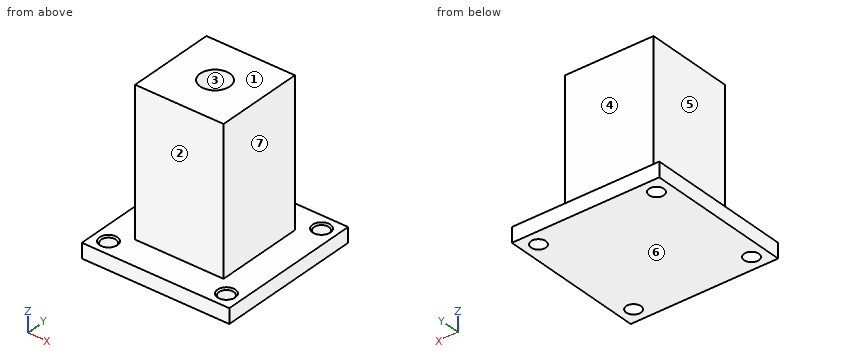
```python
from build123d import *

# Parameters (mm, degrees)
SKETCH_1_W                   = 30
SKETCH_1_H                   = 30
EXTRUDE_1_DEPTH              = 54
SKETCH_2_W                   = 50
SKETCH_2_H                   = 50
EXTRUDE_2_DEPTH              = 5
HOLE_WIZARD_M6_1_D           = 5
HOLE_WIZARD_M6_1_DEPTH       = 13.497848452
HOLE_WIZARD_M6_1_CSINK_D     = 6.05
HOLE_WIZARD_M6_1_CSINK_ANGLE = 90
HOLE_WIZARD_M6_1_TIP         = 1.502151548
SKETCH_6_R                   = 5
CUT_EXTRUDE_1_DEPTH          = 39


with BuildPart() as part:
    # 草图1 → 凸台-拉伸1 (new body)
    with BuildSketch(Plane.XY):
        with Locations((-50, 0)):
            Rectangle(SKETCH_1_W, SKETCH_1_H)
    extrude(amount=EXTRUDE_1_DEPTH)

    # 草图2 → 凸台-拉伸2 (add)
    with BuildSketch(Plane.XY):
        with Locations((-50, 0)):
            Rectangle(SKETCH_2_W, SKETCH_2_H)
    extrude(amount=EXTRUDE_2_DEPTH)

    # M6 螺纹孔1
    with Locations(Plane.XY.offset(5)):
        with Locations((-30, 20), (-70, 20), (-70, -20), (-30, -20)):
            CounterSinkHole(HOLE_WIZARD_M6_1_D / 2, HOLE_WIZARD_M6_1_CSINK_D / 2, depth=HOLE_WIZARD_M6_1_DEPTH, counter_sink_angle=HOLE_WIZARD_M6_1_CSINK_ANGLE)
            with Locations((0, 0, -(HOLE_WIZARD_M6_1_DEPTH + HOLE_WIZARD_M6_1_TIP / 2))):  # 118° drill point
                Cone(0, HOLE_WIZARD_M6_1_D / 2, HOLE_WIZARD_M6_1_TIP, mode=Mode.SUBTRACT)

    # 草图6 → 切除-拉伸1 (cut)
    with BuildSketch(Plane.XY.offset(54)):
        with Locations((-50, 0)):
            Circle(SKETCH_6_R)
    extrude(amount=-CUT_EXTRUDE_1_DEPTH, mode=Mode.SUBTRACT)


solid = part.part
```
Input: part model. Units: mm. Frame: model coordinates. Face numbers are marked on the shaded views. A direction names the side the tool comes from. Round coordinates to 2 decimals unless told otherwise and drop trailing zeros. Write each loop counter-clockwise with the first axis right and the second up, starting at its lowest first coordinate (ties: lowest second). Pieces come first, ordered by that corner, then holes. Notation, with made-up numbers: (28, 12) - (36, 12) arc R12 cw to (36, 20) - close; hole circle Ø8 at (-30.5, 41.5). An arc over 180 degrees is marked (long way). Write item = value, one per line.
(1) Section query D-D on y = 0. Output: boundary loops of the cut face in (x, z).
Geometry check:
outline = (-75, 0) - (-25, 0) - (-25, 5) - (-35, 5) - (-35, 54) - (-45, 54) - (-45, 15) - (-55, 15) - (-55, 54) - (-65, 54) - (-65, 5) - (-75, 5) - close
(2) Material intervals for probe 1 along X at (y, z) = (20, 2.25); probe 2 along Y at (x, z) = (-70, 3.35); probe 3 along Y at (x, z) = (-50, 42.5), sorted ascending.
Geometry check:
probe_1 = -75 to -72.5, -67.5 to -32.5, -27.5 to -25
probe_2 = -25 to -22.5, -17.5 to 17.5, 22.5 to 25
probe_3 = -15 to -5, 5 to 15
(3) Section query A-A on x = -30. Output: boundary loops of the cut face in (y, z) (3 decimals).
Geometry check:
outline = (-25, 0) - (-22.5, 0) - (-22.5, 4.475) - (-23.025, 5) - (-25, 5) - close; (-17.5, 0) - (17.5, 0) - (17.5, 4.475) - (16.975, 5) - (-16.975, 5) - (-17.5, 4.475) - close; (22.5, 0) - (25, 0) - (25, 5) - (23.025, 5) - (22.5, 4.475) - close
(4) Pull-direction query (Y, two-part tool) for the marked faces 1, 2 and 3; classes: +Y half, -Y half, draft (parallel to the pull), parting line (faces both ways), or undercut.
Geometry check:
face_1 = draft
face_2 = -Y half
face_3 = undercut
(5) Section query C-C on z = 31.5. Output: boundary loops of the cut face in (x, y), then the cut area to 3 significant figures.
Geometry check:
outline = (-65, -15) - (-35, -15) - (-35, 15) - (-65, 15) - close; hole circle Ø10 at (-50, 0)
area = 821 mm^2
(6) Contact query for flat-ended pins moving along their axis: pin 1 Ø24 at (x, z) = (-56.5, 32) entering from -Y; pin 2 Ø1 at (y, z) = (7, 17) entering from -X; pin 3 Ø1 at (x, z) = (-49, 40) entering from +Y; pin 4 Ø4 at (x, y) = (-30, -20) entering from -Z. Output: stop coordinate, or through.
Geometry check:
pin_1 = -15
pin_2 = -65
pin_3 = 15
pin_4 = through
(7) Section query B-B on y = 20. Output: boundary loops of the cut face in (x, z) (3 decimals).
Geometry check:
outline = (-75, 0) - (-72.5, 0) - (-72.5, 4.475) - (-73.025, 5) - (-75, 5) - close; (-67.5, 0) - (-32.5, 0) - (-32.5, 4.475) - (-33.025, 5) - (-66.975, 5) - (-67.5, 4.475) - close; (-27.5, 0) - (-25, 0) - (-25, 5) - (-26.975, 5) - (-27.5, 4.475) - close
(8) Access query for the marked faces 4, 5, 6 and 7. Directions: +Z, -Z, +X, -X, +Y, -Y. A direction counts if a zero-diameter tool reaches every point of the face in a straight line with its end or side. Return the directions, or none.
Geometry check:
face_4 = +Z, +X, -X, +Y
face_5 = +Z, -X, +Y, -Y
face_6 = -Z, +X, -X, +Y, -Y
face_7 = +Z, +X, +Y, -Y
